from build123d import *

# Parameters (mm, degrees)
SKETCH_1_4_R        = 6
BOSS_EXTRUDE1_DEPTH = 18
SKETCH_1_3_R        = 10
SKETCH_1_3_R_2      = 6
BOSS_EXTRUDE2_DEPTH = 8
SKETCH_1_4_2_R      = 12
SKETCH_1_4_2_R_2    = 10
BOSS_EXTRUDE3_DEPTH = 4
CHAMFER1_SIZE       = 0.5


with BuildPart() as part:
    # Sketch 1_4 → Boss-Extrude1 (new body)
    with BuildSketch(Plane.XY):
        Circle(SKETCH_1_4_R)
    extrude(amount=BOSS_EXTRUDE1_DEPTH)

    # 草图1<3> → Boss-Extrude2 (add)
    with BuildSketch(Plane.XY):
        Circle(SKETCH_1_3_R)
        Circle(SKETCH_1_3_R_2, mode=Mode.SUBTRACT)
    extrude(amount=BOSS_EXTRUDE2_DEPTH)

    # Sketch 1_4 2 → Boss-Extrude3 (add)
    with BuildSketch(Plane.XY):
        Circle(SKETCH_1_4_2_R)
        Circle(SKETCH_1_4_2_R_2, mode=Mode.SUBTRACT)
    extrude(amount=BOSS_EXTRUDE3_DEPTH)

    # Chamfer1
    chamfer1_edges = [part.edges().sort_by_distance(p)[0] for p in [
        (-12, 0, 0),
    ]]
    chamfer(chamfer1_edges, length=CHAMFER1_SIZE)


solid = part.part
Build history of the part. All positions in model axes, mm. A direction names the side the tool comes from. Round coordinates to 2 decimals unless told otherwise and drop trailing zeros. Write each loop counter-clockwise with the first axis right and the second up, starting at its lowest first coordinate (ties: lowest second). Pieces come first, ordered by that corner, then holes. Notation, with made-up numbers: M 30.25,-29 L 45.25,-29 A17 cw 45.25,-4 Z; hole C -22.5,78.5 d3. An arc over 180 degrees is marked long. Use CSV: the item, a comma, the result in double quotes.
1. Saw through at D-D (z = 3.25). Give the cut face in (x, y), plus the area to 3 significant figures.
Reply:
outline,"C 0,0 d24"
area,"452 mm²"
2. Tool access for faces 1 (the face through (-11.99, 0.53, 2.23)), 2 (the face through (0, -7, 8)): list every direction of +Z, -Z, +X, -X, +Y, -Y with a clear straight run to the whole face (end or side of a thin tool).
Reply:
face 1,"+Z, -Z"
face 2,"+Z"
3. Flat gauge pins, fed straight in: pin 1 (8 mm diameter, centred on x = 2.5, z = 14, fed in from +Y); pin 2 (1.5 mm diameter, centred on y = 8, z = 8, fed in from +X); pin 3 (2 mm diameter, centred on x = -9, y = 8.5, fed in from +Z). Where does each tip first touch, or does it go through?
Reply:
pin 1,"stops at y = 6"
pin 2,"stops at x = 6.89"
pin 3,"stops at z = 4"
4. Wall check: probe 1 along Z at (x, y) = (-1.75, 7); probe 2 along Z at (x, y) = (9, 6.5); probe 3 along X at (y, z) = (-3.5, 12). Give the ranges that are in metal, low to high. Write a range as from..to.
Reply:
probe 1,"z = 0..8"
probe 2,"z = 0..4"
probe 3,"x = -4.87..4.87"
5. Saw through at A-A (x = 0). Give the cut face in (y, z), plus the area to 3 significant figures.
Reply:
outline,"M -12,0.5 L -11.5,0 L 11.5,0 L 12,0.5 L 12,4 L 10,4 L 10,8 L 6,8 L 6,18 L -6,18 L -6,8 L -10,8 L -10,4 L -12,4 Z"
area,"296 mm²"
6. Saw through at C-C (z = 12.5). Give the cut face in (x, y).
Reply:
outline,"C 0,0 d12"
